```python
from build123d import *

# Parameters (mm, degrees)
SKETCH1_R           = 35
BOSS_EXTRUDE1_DEPTH = 10


with BuildPart() as part:
    # Sketch1 → Boss-Extrude1 (new body)
    with BuildSketch(Plane.XY):
        with BuildLine():
            Line((10, 0), (56, 0))
            ThreePointArc((56, 0), (96, 40), (136, 0))
            Line((136, 0), (182, 0))
            Line((182, 0), (192, 10))
            Line((192, 10), (192, 180))
            Line((192, 180), (182, 190))
            Line((182, 190), (136, 190))
            ThreePointArc((136, 190), (96, 150), (56, 190))
            Line((56, 190), (10, 190))
            Line((10, 190), (0, 180))
            Line((0, 180), (0, 10))
            Line((0, 10), (10, 0))
        make_face()
        with Locations((48, 95)):
            Circle(SKETCH1_R, mode=Mode.SUBTRACT)
        with Locations((144, 95)):
            Circle(SKETCH1_R, mode=Mode.SUBTRACT)
    extrude(amount=BOSS_EXTRUDE1_DEPTH)


solid = part.part
```
Build history of the part. All positions in model axes, mm. Round coordinates to 2 decimals unless told otherwise and drop trailing zeros. Write each loop counter-clockwise with the first axis right and the second up, starting at its lowest first coordinate (ties: lowest second). Pieces come first, ordered by that corner, then holes.
1) Mould opens along X. For faces 1 (the cylindrical face through (96.88, 150.01, 4.93)), 2 (the flat face through (33, 190, 5)), 3 (the flat face through (5, 185, 5)) say: +X half, -X half, draft (parallel to the pull), parting line (faces both ways), or undercut.
2) Band-saw the part on C-C, the plane z = 5. List the corners of the cut face in (x, y), and give its area (3 significant figures).
3) Band-saw the part on D-D, the plane x = 67. List the corners of the cut face in (y, z).
4) Pin check, flat tips, straight feed: pin 1 (1 mm diameter, centred on x = 60.5, z = 7, fed in from +Y); pin 2 (1 mm diameter, centred on x = 66, z = 6, fed in from -Y); pin 3 (1.5 mm diameter, centred on x = 115, z = 1.5, fed in from +Y). Stop position of each tip, or through.
5) Band-saw the part on A-A, the plane x = 144. List the corners of the cut face in (y, z), and give its area (3 significant figures).
6) Drill centre lines: probe 1 along X at (y, z) = (95.5, 8.75); probe 2 along Y at (x, z) = (144.5, 6.25); probe 3 along X at (y, z) = (84.5, 1.25). Where is each one in solid material? Low to high.
7) Band-saw the part on B-B, the plane y = 95. List the corners of the cut face in (x, z), and give its area (3 significant figures).
Ans:
1. face 1: undercut
1. face 2: draft
1. face 3: -X half
2. outline: (0, 10) - (10, 0) - (56, 0) arc R40 cw to (136, 0) - (182, 0) - (192, 10) - (192, 180) - (182, 190) - (136, 190) arc R40 cw to (56, 190) - (10, 190) - (0, 180) - close; hole circle Ø70 at (48, 95); hole circle Ø70 at (144, 95)
2. area: 23,600 mm2
3. outline: (27.55, 0) - (65.61, 0) - (65.61, 10) - (27.55, 10) - close; (124.39, 0) - (162.45, 0) - (162.45, 10) - (124.39, 10) - close
4. pin 1: stops at y = 172.56
4. pin 2: stops at y = 25.88
4. pin 3: stops at y = 155.22
5. outline: (0, 0) - (60, 0) - (60, 10) - (0, 10) - close; (130, 0) - (190, 0) - (190, 10) - (130, 10) - close
5. area: 1,200 mm2
6. probe 1: x = 0 to 13, 83 to 109, 179 to 192
6. probe 2: y = 0 to 60, 130 to 190
6. probe 3: x = 0 to 14.61, 81.39 to 110.61, 177.39 to 192
7. outline: (0, 0) - (13, 0) - (13, 10) - (0, 10) - close; (83, 0) - (109, 0) - (109, 10) - (83, 10) - close; (179, 0) - (192, 0) - (192, 10) - (179, 10) - close
7. area: 520 mm2
